```python
from build123d import *

# Parameters (mm, degrees)
SKETCH_1_W                = 180
SKETCH_1_H                = 190
EXTRUDE_1_DEPTH           = 10
HOLE_WIZARD_1_D           = 5.5
HOLE_WIZARD_1_CBORE_D     = 10
HOLE_WIZARD_1_CBORE_DEPTH = 5.7
PATTERN_LINEAR_1_COUNT    = 2
PATTERN_LINEAR_1_PITCH    = 94
SKETCH_4_W                = 12.05
SKETCH_4_H                = 150
CUT_EXTRUDE_1_DEPTH       = 1
SKETCH_6_R                = 2
CUT_EXTRUDE_2_DEPTH       = 1
HOLE_WIZARD_M5_1_D        = 4.2
HOLE_WIZARD_M5_1_DEPTH    = 14
HOLE_WIZARD_M5_1_TIP      = 1.2618073
FILLET_1_R                = 10
HOLE_WIZARD_M5_2_D        = 4.2
HOLE_WIZARD_M5_3_D        = 4.2
HOLE_WIZARD_6_0_6_1_D     = 6
HOLE_WIZARD_6_0_6_1_DEPTH = 10
HOLE_WIZARD_6_0_6_1_TIP   = 1.802581857
HOLE_WIZARD_M3_1_D        = 2.5


with BuildPart() as part:
    # 草图1 → 凸台-拉伸1 (new body)
    with BuildSketch(Plane.XY):
        with Locations((0, -95)):
            Rectangle(SKETCH_1_W, SKETCH_1_H)
    extrude(amount=EXTRUDE_1_DEPTH)

    # 打孔尺寸(%根据)开槽圆柱头螺钉的类型1 (through all)
    with Locations(Plane.XY.offset(10)):
        with Locations((65, -10), (3, -10)):
            hole_wizard_1 = CounterBoreHole(HOLE_WIZARD_1_D / 2, HOLE_WIZARD_1_CBORE_D / 2, HOLE_WIZARD_1_CBORE_DEPTH)

    # 阵列(线性)1: 打孔尺寸(%根据)开槽圆柱头螺钉的类型1 ×2
    with Locations(*[(0, -i * PATTERN_LINEAR_1_PITCH, 0) for i in range(1, PATTERN_LINEAR_1_COUNT)]):
        add(hole_wizard_1, mode=Mode.SUBTRACT)

    # 草图4 → 切除-拉伸1 (cut)
    with BuildSketch(Plane.XY.offset(10)):
        with Locations((-78.975, -110)):
            Rectangle(SKETCH_4_W, SKETCH_4_H)
        with Locations((-28.975, -110)):
            Rectangle(SKETCH_4_W, SKETCH_4_H)
    extrude(amount=-CUT_EXTRUDE_1_DEPTH, mode=Mode.SUBTRACT)

    # 草图6 → 切除-拉伸2 (cut)
    with BuildSketch(Plane.XY.offset(10)):
        with Locations((-72.95, -35)):
            Circle(SKETCH_6_R)
        with Locations((-85, -35)):
            Circle(SKETCH_6_R)
        with Locations((-85, -185)):
            Circle(SKETCH_6_R)
        with Locations((-72.95, -185)):
            Circle(SKETCH_6_R)
        with Locations((-35, -185)):
            Circle(SKETCH_6_R)
        with Locations((-22.95, -185)):
            Circle(SKETCH_6_R)
        with Locations((-35, -35)):
            Circle(SKETCH_6_R)
        with Locations((-22.95, -35)):
            Circle(SKETCH_6_R)
    extrude(amount=-CUT_EXTRUDE_2_DEPTH, mode=Mode.SUBTRACT)

    # M5 螺纹孔1
    with Locations(Plane(origin=(0, 0, 0), x_dir=(1, 0, 0), z_dir=(0, 1, 0))):
        with Locations((-23.975, -5), (-83.975, -5)):
            Hole(HOLE_WIZARD_M5_1_D / 2, depth=HOLE_WIZARD_M5_1_DEPTH)
            with Locations((0, 0, -(HOLE_WIZARD_M5_1_DEPTH + HOLE_WIZARD_M5_1_TIP / 2))):  # 118° drill point
                Cone(0, HOLE_WIZARD_M5_1_D / 2, HOLE_WIZARD_M5_1_TIP, mode=Mode.SUBTRACT)

    # 圆角1
    fillet_1_edges = [part.edges().sort_by_distance(p)[0] for p in [
        (90, -190, 5),
        (-90, -190, 5),
    ]]
    fillet(fillet_1_edges, radius=FILLET_1_R)

    # M5 螺纹孔2 (through all)
    with Locations(Plane.XY.offset(10)):
        with Locations((-66.95, -185), (-41, -185)):
            Hole(HOLE_WIZARD_M5_2_D / 2)

    # M5 螺纹孔3 (through all)
    with Locations(Plane.XY.offset(10)):
        with Locations((79.379496826, -119.666387024), (17.670502343, -119.666387024), (17.670502343, -89.666387024), (79.379496826, -89.666387024), (79.379496826, -25.666387024), (17.670502343, -25.666387024)):
            Hole(HOLE_WIZARD_M5_3_D / 2)

    # Ø6.0 (6) 直径孔1
    with Locations(Plane.XY.offset(10)):
        with Locations((34, -104), (34, -10)):
            Hole(HOLE_WIZARD_6_0_6_1_D / 2, depth=HOLE_WIZARD_6_0_6_1_DEPTH)
            with Locations((0, 0, -(HOLE_WIZARD_6_0_6_1_DEPTH + HOLE_WIZARD_6_0_6_1_TIP / 2))):  # 118° drill point
                Cone(0, HOLE_WIZARD_6_0_6_1_D / 2, HOLE_WIZARD_6_0_6_1_TIP, mode=Mode.SUBTRACT)

    # M3 螺纹孔1 (through all)
    with Locations(Plane.XY.offset(10)):
        with Locations((-28.975, -64.7), (-78.975, -64.7), (-78.975, -89.7), (-78.975, -114.7), (-78.975, -164.7), (-78.975, -139.7), (-28.975, -164.7), (-28.975, -139.7), (-28.975, -114.7), (-28.975, -89.7)):
            Hole(HOLE_WIZARD_M3_1_D / 2)


solid = part.part
```
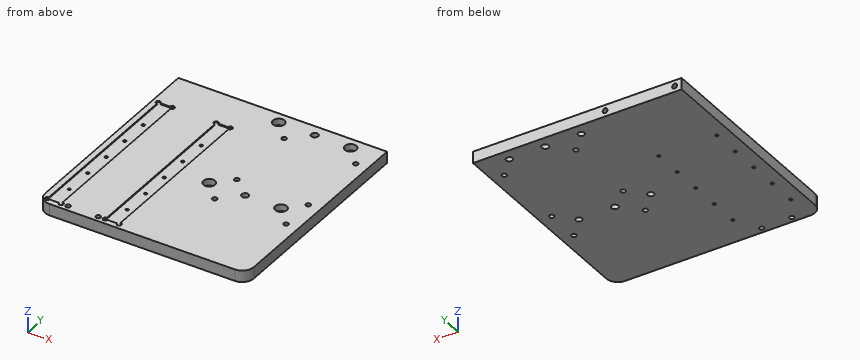
Could you check a few things on this model? Use its own coordinates, in mm. Round coordinates to 2 decimals unless told otherwise and drop trailing zeros. Write each loop counter-clockwise with the first axis right and the second up, starting at its lowest first coordinate (ties: lowest second). Pieces come first, ordered by that corner, then holes. Notation, with made-up numbers: M 26,-17 L 83,-17 A13 cw 83,-12 Z; hole C -18,74 d4. An arc over 180 degrees is marked long. Write each question's results on one line, items separated by ' | '. Start each with the question number.
1. I need wall thicknesses on L1, parallel to X at y = -94.5, z = 9.75; L2, parallel to Y at x = 65, z = 7; L3, parallel to X at y = -185, z = 7. Which ranges of each line are inside material? Lowest first, please. Write a range as from..to.
2. Imagine slicing it at A-A on x = 3. List the corners of the cut face in (y, z) for me, and give its area (3 significant figures).
3. I'm going to push flat-ended pins straight in: pin 1 Ø1.5 at (x, y) = (-9, -67) entering from -Z; pin 2 Ø3 at (x, y) = (-35, -35) entering from +Z; pin 3 Ø2.5 at (x, z) = (-83.975, 5) entering from -Y. Where does each tip first touch, or does it pass through?
Result sheet:
1) L1: x = -90..-85, -72.95..-35, -22.95..90 | L2: y = -190..-109, -99..-15, -5..0 | L3: x = -88.66..-69.05, -64.85..-43.1, -38.9..88.66
2) outline: M -190,0 L -106.75,0 L -106.75,4.3 L -109,4.3 L -109,10 L -190,10 Z; M -101.25,0 L -12.75,0 L -12.75,4.3 L -15,4.3 L -15,10 L -99,10 L -99,4.3 L -101.25,4.3 Z; M -7.25,0 L 0,0 L 0,10 L -5,10 L -5,4.3 L -7.25,4.3 Z | area: 1,740 mm^2
3) pin 1: stops at z = 0 | pin 2: stops at z = 9 | pin 3: stops at y = -189.62
